from build123d import *

# Parameters (mm, degrees)
EXTRUDE_1_DEPTH = 2317


with BuildPart() as part:
    # 草图1 → 凸台-拉伸1 (new body)
    with BuildSketch(Plane.XY):
        Polygon((7.255126662, 0), (3.255126662, 0), (3.255126662, -8.686153846), (-0.244873338, -8.686153846), (-0.244873338, 0), (-1.244873338, 0), (-1.244873338, -18.4), (-0.244873338, -18.4), (-0.244873338, -10.686153846), (3.255126662, -10.686153846), (3.255126662, -18.686153846), (4.255126662, -18.686153846), (4.255126662, -0.786153846), (7.255126662, -0.786153846), align=None)
    extrude(amount=EXTRUDE_1_DEPTH)


solid = part.part
Work out the finished part from the listing and answer in its coordinate system (mm). Give positions to 0.01 mm unless a question says otherwise; leave off trailing zeros. Loops run counter-clockwise (first coordinate to the right, second up) from the corner with the lowest first, then second, coordinate; pieces in that order, holes last. Notation, with made-up numbers: (50.25, -30) -> (82.25, -30) arc R25 ccw to (82.25, -8) -> close; hole circle Ø2 at (-27, 87). An arc over 180 degrees is marked (long way). Use a Markdown table: item, result. Add a question column.
1) Consider line 1 along X through (y, z) = (-3.25, 703.5); line 2 along Y through (x, z) = (4.75, 596.5); line 3 along Y through (x, z) = (2, 1175). Determine where each line is inside the solid, lowest interval first.
2) The part is cut by section B-B, the plane z = 1697.5. Determine the outline of the cut face in (x, y), plus the area to 3 significant figures.
3) Each of these flat-tipped pins is pushed along its axis until it touches: P1, Ø1, axis at x = 1, z = 710, coming from the +Y side; P2, Ø1.8, axis at x = 2, z = 1460, coming from the -Y side; P3, Ø3, axis at x = 1.5, y = -3, coming from the +Z side; P4, Ø9, axis at y = -10.5, z = 1108.5, coming from the +X side. Where does it stop, or does it pass through?
4) The part is cut by section C-C, the plane x = 1.75. Determine the outline of the cut face in (y, z).
5) The part is cut by section A-A, the plane y = -3.75. Determine the outline of the cut face in (x, z), plus the area to 3 significant figures.
Reported:
| question | item | result |
|---|---|---|
| 1 | line 1 | x = -1.24 to -0.24, 3.26 to 4.26 |
| 1 | line 2 | y = -0.79 to 0 |
| 1 | line 3 | y = -10.69 to -8.69 |
| 2 | outline | (-1.24, -18.4) -> (-0.24, -18.4) -> (-0.24, -10.69) -> (3.26, -10.69) -> (3.26, -18.69) -> (4.26, -18.69) -> (4.26, -0.79) -> (7.26, -0.79) -> (7.26, 0) -> (3.26, 0) -> (3.26, -8.69) -> (-0.24, -8.69) -> (-0.24, 0) -> (-1.24, 0) -> close |
| 2 | area | 46.4 mm^2 |
| 3 | P1 | stops at y = -8.69 |
| 3 | P2 | stops at y = -10.69 |
| 3 | P3 | passes through |
| 3 | P4 | stops at x = 4.26 |
| 4 | outline | (-10.69, 0) -> (-8.69, 0) -> (-8.69, 2317) -> (-10.69, 2317) -> close |
| 5 | outline | (-1.24, 0) -> (-0.24, 0) -> (-0.24, 2317) -> (-1.24, 2317) -> close; (3.26, 0) -> (4.26, 0) -> (4.26, 2317) -> (3.26, 2317) -> close |
| 5 | area | 4,630 mm^2 |
